from build123d import *

# Parameters (mm, degrees)
SKETCH_1_W                   = 85
SKETCH_1_H                   = 45
EXTRUDE_1_DEPTH              = 15
HOLE_WIZARD_M6_1_D           = 6.6
HOLE_WIZARD_M6_1_CBORE_D     = 11
HOLE_WIZARD_M6_1_CBORE_DEPTH = 6.4
SKETCH_4_R                   = 3.25
CUT_EXTRUDE_1_DEPTH          = 162
CHAMFER_1_SIZE               = 3


with BuildPart() as part:
    # 草图1 → 凸台-拉伸1 (new body)
    with BuildSketch(Plane.XY):
        Rectangle(SKETCH_1_W, SKETCH_1_H)
        with BuildLine():
            Line((-25, 7.5), (25, 7.5))
            ThreePointArc((25, 7.5), (32.5, 0), (25, -7.5))
            Line((25, -7.5), (-25, -7.5))
            ThreePointArc((-25, -7.5), (-32.5, 0), (-25, 7.5))
        make_face(mode=Mode.SUBTRACT)
    extrude(amount=EXTRUDE_1_DEPTH)

    # M6 六角凹头螺钉的柱形沉头孔1 (through all)
    with Locations(Plane.XY.offset(15)):
        with Locations((-34.5, 12), (-34.5, -12), (34.5, -12), (34.5, 12)):
            CounterBoreHole(HOLE_WIZARD_M6_1_D / 2, HOLE_WIZARD_M6_1_CBORE_D / 2, HOLE_WIZARD_M6_1_CBORE_DEPTH)

    # 草图4 → 切除-拉伸1 (cut)
    with BuildSketch(Plane.ZY.offset(42.5)):
        with Locations((7.5, 0)):
            Circle(SKETCH_4_R)
    extrude(amount=-CUT_EXTRUDE_1_DEPTH, mode=Mode.SUBTRACT)

    # 倒角1
    chamfer_1_edges = [part.edges().sort_by_distance(p)[0] for p in [
        (42.5, -22.5, 7.5),
        (-42.5, -22.5, 7.5),
        (-42.5, 22.5, 7.5),
        (42.5, 22.5, 7.5),
    ]]
    chamfer(chamfer_1_edges, length=CHAMFER_1_SIZE)


solid = part.part
Read the model definition and answer for the solid it produces. Units are mm, in the model's axes. A direction names the side the tool comes from. Coordinates: 2 decimals unless noted, no trailing zeros. Write each loop counter-clockwise with the first axis right and the second up, starting at its lowest first coordinate (ties: lowest second). Pieces come first, ordered by that corner, then holes. Notation, with made-up numbers: (-25, 68.25) -> (32, 68.25) arc R15 ccw to (32, 88.25) -> close; hole circle Ø9 at (53, -27.5). An arc over 180 degrees is marked (long way). Return JSON: item names as keys, results as strings.
(1) The part is cut by section A-A on z = 7.5. Give the vertices of the cut face in (x, y).
Answers below:
{"outline": "(-42.5, -19.5) -> (-39.5, -22.5) -> (39.5, -22.5) -> (42.5, -19.5) -> (42.5, -3.25) -> (31.76, -3.25) arc R7.5 cw to (25, -7.5) -> (-25, -7.5) arc R7.5 cw to (-31.76, -3.25) -> (-42.5, -3.25) -> close; (-42.5, 3.25) -> (-31.76, 3.25) arc R7.5 cw to (-25, 7.5) -> (25, 7.5) arc R7.5 cw to (31.76, 3.25) -> (42.5, 3.25) -> (42.5, 19.5) -> (39.5, 22.5) -> (-39.5, 22.5) -> (-42.5, 19.5) -> close; hole circle Ø6.6 at (-34.5, -12); hole circle Ø6.6 at (-34.5, 12); hole circle Ø6.6 at (34.5, -12); hole circle Ø6.6 at (34.5, 12)"}
(2) The part is cut by section D-D on z = 3. Give the vertices of the cut face in (x, y), then the cut area to 3 significant figures.
Answers below:
{"outline": "(-42.5, -19.5) -> (-39.5, -22.5) -> (39.5, -22.5) -> (42.5, -19.5) -> (42.5, 19.5) -> (39.5, 22.5) -> (-39.5, 22.5) -> (-42.5, 19.5) -> close; hole circle Ø6.6 at (-34.5, -12); hole circle Ø6.6 at (-34.5, 12); hole (-25, -7.5) -> (25, -7.5) arc R7.5 ccw to (25, 7.5) -> (-25, 7.5) arc R7.5 ccw to start; hole circle Ø6.6 at (34.5, -12); hole circle Ø6.6 at (34.5, 12)", "area": "2,740 mm^2"}
(3) For a pull along Y with two mould halves and no side action, classify faces 1 (the flat face through (-1, 22.5, 7)), 2 (the flat face through (-35, -16, 8.6)), 3 (the flat face through (-42.5, 0, 4)) as pulls with the +Y half, pulls with the -Y half, needs draft (parallel to the pull), parting line crosses it, or undercut.
Answers below:
{"face 1": "pulls with the +Y half", "face 2": "undercut", "face 3": "needs draft"}
(4) This flat-tipped pin is pushed along its axis until it touches: P1, Ø10.5, axis at x = -34.5, y = 12, coming from the +Z side. Where does it stop, or does it pass through?
Answers below:
{"P1": "z = 8.6"}
(5) Which of the six approach directions +Z, -Z, +X, -X, +Y, -Y give full straight-line access (tool end or side, diameter ignored) to faces 4 (the flat face through (-35, 8, 8.6)), 5 (the flat face through (-41, -21, 7)), 6 (the cylindrical face through (32.5, 0.16, 4.06))?
Answers below:
{"face 4": "+Z", "face 5": "+Z, -Z, -X, -Y", "face 6": "+Z, -Z"}
(6) The part is cut by section B-B on y = 12. Give the vertices of the cut face in (x, z), then the cut area to 3 significant figures.
Answers below:
{"outline": "(-42.5, 0) -> (-37.8, 0) -> (-37.8, 8.6) -> (-40, 8.6) -> (-40, 15) -> (-42.5, 15) -> close; (-31.2, 0) -> (31.2, 0) -> (31.2, 8.6) -> (29, 8.6) -> (29, 15) -> (-29, 15) -> (-29, 8.6) -> (-31.2, 8.6) -> close; (37.8, 0) -> (42.5, 0) -> (42.5, 15) -> (40, 15) -> (40, 8.6) -> (37.8, 8.6) -> close", "area": "1,020 mm^2"}
(7) Consider line 1 along Y through (x, z) = (34.5, 3.75); line 2 along Y through (x, z) = (-34.5, 11.5); line 3 along Y through (x, z) = (8, 12.25). Determine where each line is inside the solid, lowest interval first. Write a range as from..to.
Answers below:
{"line 1": "-22.5..-15.3, -8.7..8.7, 15.3..22.5", "line 2": "-22.5..-17.5, -6.5..6.5, 17.5..22.5", "line 3": "-22.5..-7.5, 7.5..22.5"}
(8) The part is cut by section C-C on x = 34.5. Give the vertices of the cut face in (y, z).
Answers below:
{"outline": "(-22.5, 0) -> (-15.3, 0) -> (-15.3, 8.6) -> (-17.5, 8.6) -> (-17.5, 15) -> (-22.5, 15) -> close; (-8.7, 0) -> (8.7, 0) -> (8.7, 8.6) -> (6.5, 8.6) -> (6.5, 15) -> (-6.5, 15) -> (-6.5, 8.6) -> (-8.7, 8.6) -> close; (15.3, 0) -> (22.5, 0) -> (22.5, 15) -> (17.5, 15) -> (17.5, 8.6) -> (15.3, 8.6) -> close; hole circle Ø6.5 at (0, 7.5)"}
